from build123d import *

# Parameters (mm, degrees)
BRACKET_BODY_DEPTH         = 25
CRADLE_SLOT_CUT_DEPTH      = 148.57032222
CRADLE_SLOT_CUT_DEPTH_BACK = 148.57032222
CRADLE_SLOT_SKETCH_W       = 42
CRADLE_SLOT_SKETCH_H       = 19
BASE_CUT_OUT_SKETCH_R      = 15
BASE_CUT_OUTS_DEPTH        = 85.083292038


with BuildPart() as part:
    # Bracket Profile Sketch → Bracket Body (new, symmetric)
    with BuildSketch(Plane.XY):
        with BuildLine():
            Line((-62, 0), (-15, 0))
            ThreePointArc((-15, 0), (0, 15), (15, 0))
            Line((15, 0), (62, 0))
            Line((62, 0), (62, 25))
            Line((62, 25), (5, 25))
            Line((5, 25), (5, 43.575714714))
            ThreePointArc((5, 43.575714714), (17.23368794, 51.325205669), (22, 65))
            Line((22, 65), (22, 76))
            Line((22, 76), (14, 76))
            Line((14, 76), (14, 65))
            ThreePointArc((14, 65), (0, 51), (-14, 65))
            Line((-14, 65), (-14, 76))
            Line((-14, 76), (-22, 76))
            Line((-22, 76), (-22, 65))
            ThreePointArc((-22, 65), (-17.23368794, 51.325205669), (-5, 43.575714714))
            Line((-5, 43.575714714), (-5, 25))
            Line((-5, 25), (-62, 25))
            Line((-62, 25), (-62, 0))
        make_face()
    extrude(amount=BRACKET_BODY_DEPTH, both=True)

    # Cradle Slot Sketch → Cradle Slot Cut (cut, two sides: drawn at the far end of the back side and taken through both)
    with BuildSketch(Plane(origin=(62, 0, 0), x_dir=(0, 0, -1), z_dir=(1, 0, 0)).offset(-CRADLE_SLOT_CUT_DEPTH_BACK)):
        with Locations((4, 9.5)):
            Rectangle(CRADLE_SLOT_SKETCH_W, CRADLE_SLOT_SKETCH_H)
    extrude(amount=CRADLE_SLOT_CUT_DEPTH + CRADLE_SLOT_CUT_DEPTH_BACK, mode=Mode.SUBTRACT)

    # Base Cut-Out Sketch → Base Cut-Outs (cut, through all)
    with BuildSketch(Plane(origin=(0, 25, 0), x_dir=(1, 0, 0), z_dir=(0, 1, 0))):
        with Locations(Location((-32, 0, 0), (0, 0, 270))):
            Circle(BASE_CUT_OUT_SKETCH_R)
        with Locations(Location((32, 0, 0), (0, 0, 270))):
            Circle(BASE_CUT_OUT_SKETCH_R)
    extrude(amount=-BASE_CUT_OUTS_DEPTH, mode=Mode.SUBTRACT)


solid = part.part
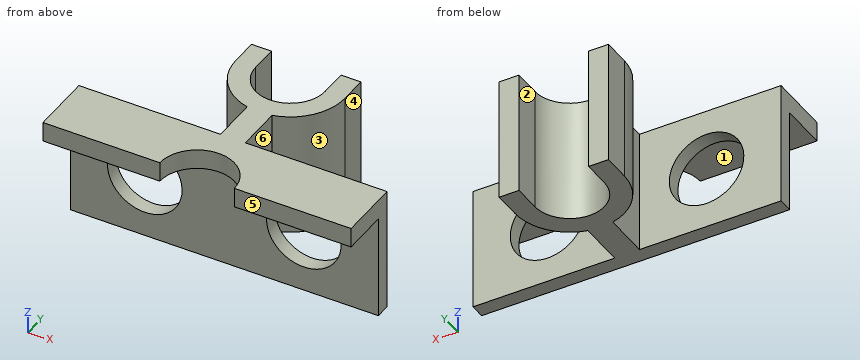
The listing builds one solid part. Answer for the finished solid, in the listing's coordinates (mm). Face numbers are marked on the shaded views. A direction names the side the tool comes from. Coordinates: 2 decimals unless noted, no trailing zeros. Loops run counter-clockwise (first coordinate to the right, second up) from the corner with the lowest first, then second, coordinate; pieces in that order, holes last. Notation, with made-up numbers: (20, 28) -> (62, 28) arc R29 cw to (62, 58) -> close; hole circle Ø1 at (2, 11.25). An arc over 180 degrees is marked (long way). Answer in a Markdown table with one row per item. Add a question column.
1. Consider line 1 (X direction, y = 21, z = 0); line 2 (X direction, y = 32, z = -11); line 3 (X direction, y = 67.5, z = -12.5). Determine where each line is inside the solid, lowest interval first. Write a range as [from, to].
2. The part is cut by section B-B, the plane y = 66.5. Write down the section's boundary in (x, z), then the cut area to 3 significant figures.
3. The part is cut by section C-C, the plane x = 32. Write down the section's boundary in (y, z).
4. For the marked faces 1, 2 and 3, determine the directions among +Z, -Z, +X, -X, +Y, -Y from which every point of the face is accessible in a straight line to the end or side of a thin tool.
5. The part is cut by section A-A, the plane z = 0. Write down the section's boundary in (x, y).
6. Flat-ended cylindrical pins translate along their axes: P1, Ø15, axis at x = -10.5, y = 9.5, coming from the -Z side; P2, Ø12, axis at y = 73, z = 11, coming from the +X side; P3, Ø12.5, axis at x = 25.5, z = -9, coming from the -Y side; P4, Ø25, axis at x = 28.5, z = 6, coming from the +Y side. Find the tip coordinate at first contact, or state that the pin passes through.
7. The part is cut by section D-D, the plane x = -19.5. Write down the section's boundary in (y, z), then the cut area to 3 significant figures.
8. Determine the mould class of the marked faces 4, 5 and 6 for opening direction Y: +Y half, -Y half, draft (parallel to the pull), parting line (faces both ways), or undercut.
Answer below:
| question | item | result |
|---|---|---|
| 1 | line 1 | [-62, -47], [-17, 17], [47, 62] |
| 1 | line 2 | [-5, 5] |
| 1 | line 3 | [-22, -14], [14, 22] |
| 2 | outline | (-22, -25) -> (-14, -25) -> (-14, 25) -> (-22, 25) -> close; (14, -25) -> (22, -25) -> (22, 25) -> (14, 25) -> close |
| 2 | area | 800 mm2 |
| 3 | outline | (0, 17) -> (19, 17) -> (19, 15) -> (25, 15) -> (25, 25) -> (0, 25) -> close; (19, -25) -> (25, -25) -> (25, -15) -> (19, -15) -> close |
| 4 | face 1 | -Z, +X, -X, -Y |
| 4 | face 2 | +Z, -Z, +Y |
| 4 | face 3 | +Z, -Z, +X |
| 5 | outline | (-62, 19) -> (-47, 19) -> (-47, 25) -> (-62, 25) -> close; (-22, 65) arc R22 ccw to (-5, 43.58) -> (-5, 25) -> (-17, 25) -> (-17, 19) -> (17, 19) -> (17, 25) -> (5, 25) -> (5, 43.58) arc R22 ccw to (22, 65) -> (22, 76) -> (14, 76) -> (14, 65) arc R14 cw to (-14, 65) -> (-14, 76) -> (-22, 76) -> close; (47, 19) -> (62, 19) -> (62, 25) -> (47, 25) -> close |
| 6 | P1 | z = 17 |
| 6 | P2 | x = 22 |
| 6 | P3 | y = 19 |
| 6 | P4 | y = 76 |
| 7 | outline | (0, 17) -> (19, 17) -> (19, 8.29) -> (25, 8.29) -> (25, 25) -> (0, 25) -> close; (19, -25) -> (25, -25) -> (25, -8.29) -> (19, -8.29) -> close; (54.81, -25) -> (76, -25) -> (76, 25) -> (54.81, 25) -> close |
| 7 | area | 1,410 mm2 |
| 8 | face 4 | draft |
| 8 | face 5 | -Y half |
| 8 | face 6 | undercut |
